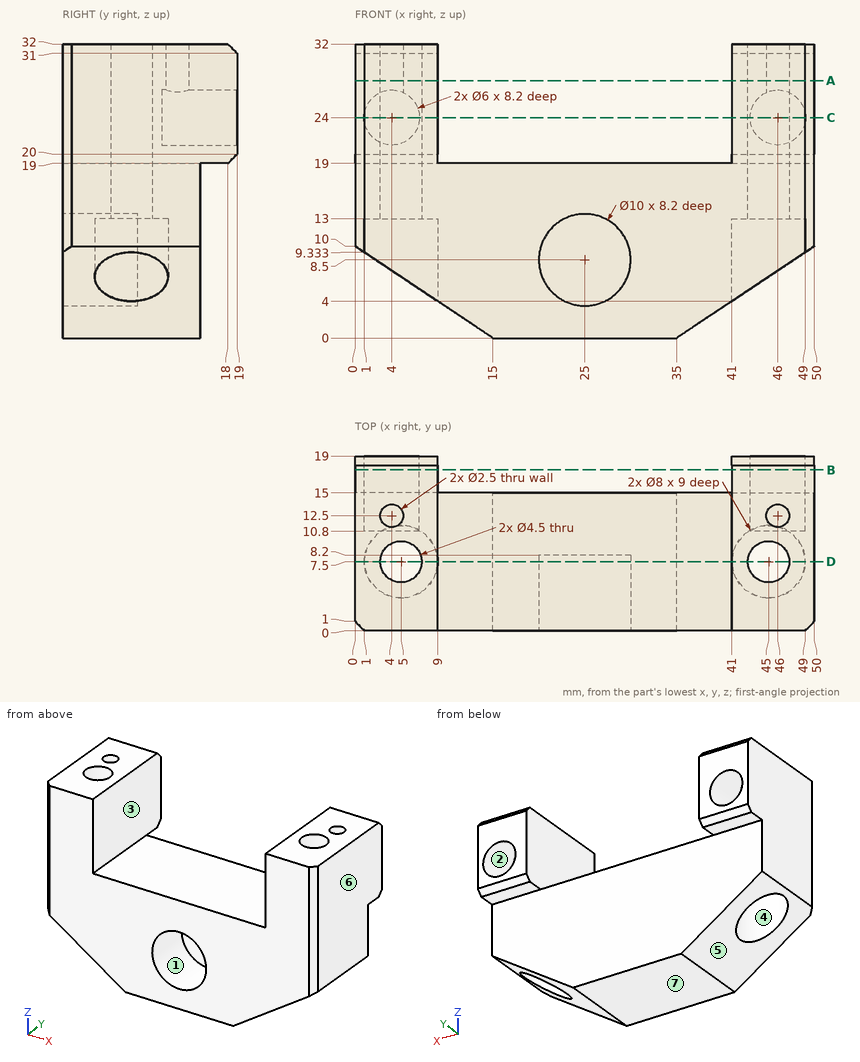
Verification items for this drawing (mm, ordinates from the low corner). A direction names the side the tool comes from. Give positions to 0.01 mm unless a question says otherwise; leave off trailing zeros. Loops run counter-clockwise (first coordinate to the right, second up) from the corner with the lowest first, then second, coordinate; pieces in that order, holes last. Notation, with made-up numbers: M 20,12.5 L 34,12.5 A29 ccw 34,46.5 Z; hole C 4.5,39 d7. An arc over 180 degrees is marked long. Answer in a Markdown table with one row per item.
1) Cross-section at A-A (z = 28). Enter the section's corners in (x, y).
Solutions:
| item | result |
|---|---|
| outline | M 0,1 L 1,0 L 9,0 L 9,19 L 0,19 Z; M 41,0 L 49,0 L 50,1 L 50,19 L 41,19 Z; hole C 5,7.5 d4.5; hole C 4,12.5 d2.5; hole C 45,7.5 d4.5; hole C 46,12.5 d2.5 |
2) Depth check by flat-ended pin: pin 1 (0.9 mm diameter, centred on x = 44, y = 17, fed in from -Z); pin 2 (1.8 mm diameter, centred on x = 47.5, z = 23.5, fed in from +Y); pin 3 (7 mm diameter, centred on x = 5, y = 7.5, fed in from -Z); pin 4 (2 mm diameter, centred on x = 17.5, y = 16.5, fed in from +Z). Enter the tip coordinate at first touch or a pass-through.
Solutions:
| item | result |
|---|---|
| pin 1 | stops at z = 19 |
| pin 2 | stops at y = 10.8 |
| pin 3 | stops at z = 13 |
| pin 4 | passes through |
3) Mould release check, pull along X, two halves, no side actions. Record for the marked faces 4, 5, 6 and 7: released by +X, released by -X, zero draft, split by the parting line, or undercut.
Solutions:
| item | result |
|---|---|
| face 4 | undercut |
| face 5 | released by -X |
| face 6 | released by +X |
| face 7 | zero draft |
4) Cross-section at D-D (y = 7.5). Enter the section's corners in (x, z), plus the area to 3 significant figures.
Solutions:
| item | result |
|---|---|
| outline | M 0,10 L 1,9.33 L 1,13 L 2.75,13 L 2.75,32 L 0,32 Z; M 7.25,13 L 9,13 L 9,4 L 15,0 L 35,0 L 41,4 L 41,13 L 42.75,13 L 42.75,32 L 41,32 L 41,19 L 9,19 L 9,32 L 7.25,32 Z; M 47.25,13 L 49,13 L 49,9.33 L 50,10 L 50,32 L 47.25,32 Z; hole C 25,8.5 d10 |
| area | 683 mm^2 |
5) Tool access check on the marked faces 1, 2 and 3. Record the directions out of +Z, -Z, +X, -X, +Y, -Y that give a thin tool (end or side, any length) a straight path to the whole face; none if there is none.
Solutions:
| item | result |
|---|---|
| face 1 | -Y |
| face 2 | +Y |
| face 3 | +Z, +Y, -Y |
6) Thickness scan on line 1 (X direction, y = 12.5, z = 27.8); line 2 (X direction, y = 15.25, z = 27.5); line 3 (Y direction, x = 5, z = 24). Record the ranges inside material, lowest first.
Solutions:
| item | result |
|---|---|
| line 1 | x = 0 to 2.75, 5.25 to 9, 41 to 44.75, 47.25 to 50 |
| line 2 | x = 0 to 9, 41 to 50 |
| line 3 | y = 0 to 5.25, 9.75 to 10.8 |
7) Cross-section at B-B (y = 17.5). Enter the section's corners in (x, z).
Solutions:
| item | result |
|---|---|
| outline | M 0,19 L 9,19 L 9,32 L 0,32 Z; M 41,19 L 50,19 L 50,32 L 41,32 Z; hole C 4,24 d6; hole C 46,24 d6 |
8) Cross-section at C-C (z = 24). Enter the section's corners in (x, y).
Solutions:
| item | result |
|---|---|
| outline | M 0,1 L 1,0 L 9,0 L 9,19 L 7,19 L 7,10.8 L 1,10.8 L 1,19 L 0,19 Z; M 41,0 L 49,0 L 50,1 L 50,19 L 49,19 L 49,10.8 L 43,10.8 L 43,19 L 41,19 Z; hole C 5,7.5 d4.5; hole C 45,7.5 d4.5 |
